```python
from build123d import *

# Parameters (mm, degrees)
SKETCH1_W           = 25
SKETCH1_H           = 25
BOSS_EXTRUDE1_DEPTH = 20
SKETCH2_R           = 4
BOSS_EXTRUDE2_DEPTH = 10


with BuildPart() as part:
    # Sketch1 → Boss-Extrude1 (new body)
    with BuildSketch(Plane(origin=(0, 0, 0), x_dir=(1, 0, 0), z_dir=(0, 1, 0))):
        Rectangle(SKETCH1_W, SKETCH1_H)
    extrude(amount=BOSS_EXTRUDE1_DEPTH)

    # Sketch2 → Boss-Extrude2 (add)
    with BuildSketch(Plane.XY.offset(12.5)):
        with Locations((0, 10)):
            Circle(SKETCH2_R)
    boss_extrude2 = extrude(amount=BOSS_EXTRUDE2_DEPTH)

    # Mirror1: Boss-Extrude2 across plane
    add(boss_extrude2.mirror(Plane.XY))


solid = part.part
```
The listing builds one solid part. Answer for the finished solid, in the listing's coordinates (mm). A direction names the side the tool comes from. Round coordinates to 2 decimals unless told otherwise and drop trailing zeros. Write each loop counter-clockwise with the first axis right and the second up, starting at its lowest first coordinate (ties: lowest second). Pieces come first, ordered by that corner, then holes. Notation, with made-up numbers: (41.25, 7) -> (87.25, 7) arc R14 cw to (87.25, 13) -> close; hole circle Ø11 at (41.25, 28.5). An arc over 180 degrees is marked (long way). Use CSV: the item, a comma, the result in double quotes. Start each with the question number.
(1) Section A-A on y = 10 is taken. Give the vertices of the cut face in (x, z), then the cut area to 3 significant figures.
(2) Section B-B on x = 0 is taken. Give the vertices of the cut face in (y, z), then the cut area to 3 significant figures.
(3) Section C-C on z = -15 is taken. Give the vertices of the cut face in (x, y), then the cut area to 3 significant figures.
(4) This flat-tipped pin is pushed along its axis until it touches: pin 1 (3 mm diameter, centred on x = -8.5, y = 15, fed in from -Z). Where does it stop, or does it pass through?
(5) Section D-D on x = -7.5 is taken. Give the vertices of the cut face in (y, z), then the cut area to 3 significant figures.
(6) Consider L1, parallel to Z at x = -6, y = 2.25; L2, parallel to X at y = 9.75, z = 17. Determine where each line is inside the solid, lowest interval first. Write a range as from..to.
(7) Which of the six approach directions +Z, -Z, +X, -X, +Y, -Y give full straight-line access (tool end or side, diameter ignored) to faces 1 (the face through (-0.521, 13.966, -17.43)), 2 (the face through (0, 10, 22.5)), 3 (the face through (0, 5, 12.5))?
A:
1,outline,"(-12.5, -12.5) -> (-4, -12.5) -> (-4, -22.5) -> (4, -22.5) -> (4, -12.5) -> (12.5, -12.5) -> (12.5, 12.5) -> (4, 12.5) -> (4, 22.5) -> (-4, 22.5) -> (-4, 12.5) -> (-12.5, 12.5) -> close"
1,area,"785 mm²"
2,outline,"(0, -12.5) -> (6, -12.5) -> (6, -22.5) -> (14, -22.5) -> (14, -12.5) -> (20, -12.5) -> (20, 12.5) -> (14, 12.5) -> (14, 22.5) -> (6, 22.5) -> (6, 12.5) -> (0, 12.5) -> close"
2,area,"660 mm²"
3,outline,"circle Ø8 at (0, 10)"
3,area,"50.3 mm²"
4,pin 1,"stops at z = -12.5"
5,outline,"(0, -12.5) -> (20, -12.5) -> (20, 12.5) -> (0, 12.5) -> close"
5,area,"500 mm²"
6,L1,"z = -12.5..12.5"
6,L2,"x = -3.99..3.99"
7,face 1,"-Z"
7,face 2,"+Z, +X, -X, +Y, -Y"
7,face 3,"+Z"
